from build123d import *

# Parameters (mm, degrees)
SKETCH1_R             = 5
BOSS_EXTRUDE1_DEPTH   = 12
SKETCH2_R             = 3
BOSS_EXTRUDE2_DEPTH   = 6.5
M4_TAPPED_HOLE1_D     = 3.3
M4_TAPPED_HOLE1_DEPTH = 10.1
M4_TAPPED_HOLE1_TIP   = 0.991420021
SKETCH5_R             = 2.5
BOSS_EXTRUDE3_DEPTH   = 9
SKETCH6_R             = 2
CUT_EXTRUDE1_DEPTH    = 7.5
CHAMFER1_SIZE         = 0.5


with BuildPart() as part:
    # Sketch1 → Boss-Extrude1 (new body)
    with BuildSketch(Plane.XY):
        Circle(SKETCH1_R)
    extrude(amount=BOSS_EXTRUDE1_DEPTH)

    # Sketch2 → Boss-Extrude2 (add)
    with BuildSketch(Plane.XY.offset(12)):
        with Locations(Location((0, 0, 0), (0, 0, 180))):
            Circle(SKETCH2_R)
    extrude(amount=BOSS_EXTRUDE2_DEPTH)

    # M4 Tapped Hole1
    with Locations(Plane.XY.offset(18.5)):
        with Locations((0, 0)):
            Hole(M4_TAPPED_HOLE1_D / 2, depth=M4_TAPPED_HOLE1_DEPTH)
            with Locations((0, 0, -(M4_TAPPED_HOLE1_DEPTH + M4_TAPPED_HOLE1_TIP / 2))):  # 118° drill point
                Cone(0, M4_TAPPED_HOLE1_D / 2, M4_TAPPED_HOLE1_TIP, mode=Mode.SUBTRACT)

    # Sketch5 → Boss-Extrude3 (add)
    with BuildSketch(Plane(origin=(0, 0, 0), x_dir=(-1, 0, 0), z_dir=(0, 0, -1))):
        with Locations(Location((0, 0, 0), (0, 0, 180))):
            Circle(SKETCH5_R)
    extrude(amount=BOSS_EXTRUDE3_DEPTH)

    # Sketch6 → Cut-Extrude1 (cut, symmetric)
    with BuildSketch(Plane(origin=(0, 0, 0), x_dir=(1, 0, 0), z_dir=(0, 1, 0))):
        with Locations(Location((0, -5, 0), (0, 0, 270))):
            Circle(SKETCH6_R)
    extrude(amount=CUT_EXTRUDE1_DEPTH, both=True, mode=Mode.SUBTRACT)

    # Chamfer1
    chamfer1_edges = [part.edges().sort_by_distance(p)[0] for p in [
        (-5, 0, 0),
        (-5, 0, 12),
    ]]
    chamfer(chamfer1_edges, length=CHAMFER1_SIZE)


solid = part.part
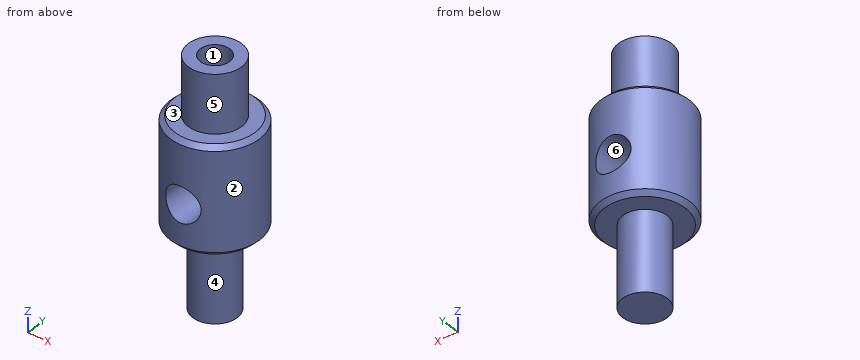
The model under review builds one solid part; all positions refer to its coordinate system, in mm. Face numbers are marked on the shaded views. A direction names the side the tool comes from. Round coordinates to 2 decimals unless told otherwise and drop trailing zeros. Order: outer loops, then holes, each group sorted by start corner. A loop starts at its lowest first (then second) coordinate and runs counter-clockwise, first axis right, second up. Notation, with made-up numbers: (66.25, 84) -> (103.25, 84) arc R11 ccw to (103.25, 89) -> close; hole circle Ø4 at (45.5, 88). An arc over 180 degrees is marked (long way). Write item = value, one per line. Start each with the question number.
Item 1: Consider section C-C on z = -2.25. Write out the cut boundary in (x, y), plus the area to 3 significant figures.
Item 2: For line 1 along Y through (x, z) = (0, 10.75); line 2 along Y through (x, z) = (0, 14.5); line 3 along Z through (x, y) = (0, -3.5), list the stretches that pass through material, from the lowest coordinate up.
Item 3: Consider section A-A on z = 12.25. Write out the cut boundary in (x, y), plus the area to 3 significant figures.
Item 4: Clearance check with flat-ended pins moving along their axes: pin 1 Ø1 at (x, z) = (2, 14.5) entering from -Y; pin 2 Ø4 at (y, z) = (1.5, -4) entering from +X; pin 3 Ø5 at (y, z) = (3.5, -3) entering from +X. State where each tip first meets the part, or that it passes through.
Item 5: Mouldability with a two-part tool opening along Y and no side actions: class the marked faces 1, 2 and 3 as released by +Y, released by -Y, zero draft, split by the parting line, or undercut.
Item 6: Consider section B-B on z = 5. Write out the cut boundary in (x, y), plus the area to 3 significant figures.
Item 7: For the marked faces 4, 5 and 6, list the 3-axis set-ups (+Z, -Z, +X, -X, +Y, -Y) from which the entire face can be reached by the end or side of a thin tool; tool diameter is ignored.
Conclusion:
q1.outline = circle Ø5 at (0, 0)
q1.area = 19.6 mm2
q2.line_1 = -5 to -1.65, 1.65 to 5
q2.line_2 = -3 to -1.65, 1.65 to 3
q2.line_3 = 0 to 3, 7 to 12
q3.outline = circle Ø6 at (0, 0); hole circle Ø3.3 at (0, 0)
q3.area = 19.7 mm2
q4.pin_1 = -2.6
q4.pin_2 = 2.5
q4.pin_3 = 2.29
q5.face_1 = undercut
q5.face_2 = split by the parting line
q5.face_3 = zero draft
q6.outline = (-2, -4.58) -> (-2, 4.58) arc R5 ccw to start; (2, -4.58) arc R5 ccw to (2, 4.58) -> close
q6.area = 39.6 mm2
q7.face_4 = -Z
q7.face_5 = +Z
q7.face_6 = +Y, -Y
